Design review of the part built by this model. Coordinates are the model's own, in mm. Coordinates: 2 decimals unless noted, no trailing zeros. Loops run counter-clockwise (first coordinate to the right, second up) from the corner with the lowest first, then second, coordinate; pieces in that order, holes last. Notation, with made-up numbers: (9, 75.25) -> (14, 75.25) arc R35 cw to (14, 107.25) -> close; hole circle Ø6 at (73.25, 44). An arc over 180 degrees is marked (long way). Answer as a JSON object with one key per item and string values.
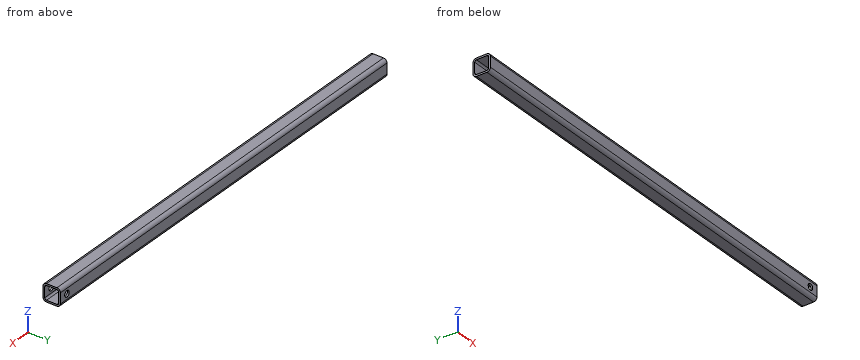
```python
from build123d import *

# Parameters (mm, degrees)
GB_6728_1986_040_X_40_X_4_1_DEPTH = 1000
HOLE_WIZARD_M16_1_D               = 14


with BuildPart() as part:
    # Sketch12 → Gb／6728-1986方形空心型钢 040 X 40 X 4(1) (new body)
    with BuildSketch(Plane.ZY):
        with BuildLine():
            Line((-12, -20), (12, -20))
            ThreePointArc((12, -20), (17.656854249, -17.656854249), (20, -12))
            Line((20, -12), (20, 12))
            ThreePointArc((20, 12), (17.656854249, 17.656854249), (12, 20))
            Line((12, 20), (-12, 20))
            ThreePointArc((-12, 20), (-17.656854249, 17.656854249), (-20, 12))
            Line((-20, 12), (-20, -12))
            ThreePointArc((-20, -12), (-17.656854249, -17.656854249), (-12, -20))
        make_face()
        with BuildLine():
            Line((-12, -16), (12, -16))
            ThreePointArc((12, -16), (14.828427125, -14.828427125), (16, -12))
            Line((16, -12), (16, 12))
            ThreePointArc((16, 12), (14.828427125, 14.828427125), (12, 16))
            Line((12, 16), (-12, 16))
            ThreePointArc((-12, 16), (-14.828427125, 14.828427125), (-16, 12))
            Line((-16, 12), (-16, -12))
            ThreePointArc((-16, -12), (-14.828427125, -14.828427125), (-12, -16))
        make_face(mode=Mode.SUBTRACT)
    extrude(amount=GB_6728_1986_040_X_40_X_4_1_DEPTH)

    # M16 螺纹孔1 (through all)
    with Locations(Plane(origin=(0, 20, 0), x_dir=(1, 0, 0), z_dir=(0, 1, 0))):
        with Locations((-20, 0)):
            Hole(HOLE_WIZARD_M16_1_D / 2)


solid = part.part
```
1) Add section A-A, the plane y = -5. Give the boundary of the cut face in (x, z).
Completed:
{"outline": "(-1000, -20) -> (0, -20) -> (0, -16) -> (-1000, -16) -> close; (-1000, 16) -> (0, 16) -> (0, 20) -> (-1000, 20) -> close"}
2) Add section C-C, the plane z = 0. Give the boundary of the cut face in (x, y).
Completed:
{"outline": "(-1000, -20) -> (-27, -20) -> (-27, -16) -> (-1000, -16) -> close; (-1000, 16) -> (-27, 16) -> (-27, 20) -> (-1000, 20) -> close; (-13, -20) -> (0, -20) -> (0, -16) -> (-13, -16) -> close; (-13, 16) -> (0, 16) -> (0, 20) -> (-13, 20) -> close"}
3) Clearance check with flat-ended pins moving along their axes: pin 1 Ø16 at (x, z) = (-20, 0) entering from -Y; pin 2 Ø3 at (x, z) = (-759, 15.5) entering from +Y; pin 3 Ø12.5 at (x, z) = (-20, 0) entering from +Y. State where each tip first meets the part, or that it passes through.
Completed:
{"pin 1": "y = -20", "pin 2": "y = 19.75", "pin 3": "through"}
4) Wall thickness on probe 1 along Z at (x, y) = (-181.5, -2.5); probe 2 along Z at (x, y) = (-20, 19): over which ranges is each line inside the solid? List them lowest first.
Completed:
{"probe 1": "-20 to -16, 16 to 20", "probe 2": "-15.87 to -7, 7 to 15.87"}
5) Add section B-B, the plane x = -668. Give the boundary of the cut face in (y, z), and give its area (3 significant figures).
Completed:
{"outline": "(-20, -12) arc R8 ccw to (-12, -20) -> (12, -20) arc R8 ccw to (20, -12) -> (20, 12) arc R8 ccw to (12, 20) -> (-12, 20) arc R8 ccw to (-20, 12) -> close; hole (-16, -12) arc R4 ccw to (-12, -16) -> (12, -16) arc R4 ccw to (16, -12) -> (16, 12) arc R4 ccw to (12, 16) -> (-12, 16) arc R4 ccw to (-16, 12) -> close", "area": "535 mm²"}
